from build123d import *

# Parameters (mm, degrees)
SKETCH1_W                  = 380
SKETCH1_H                  = 150
BOSS_EXTRUDE1_DEPTH        = 14
CHAMFER1_SIZE              = 1
SKETCH2_R                  = 20
CUT_EXTRUDE1_DEPTH         = 409.773776067
F_8_0_8_DIAMETER_HOLE1_D   = 8
LPATTERN1_COUNT            = 2
LPATTERN1_PITCH            = 270
F_13_0_13_DIAMETER_HOLE1_D = 13
M6_TAPPED_HOLE1_D          = 5
M6_TAPPED_HOLE1_DEPTH      = 15
M6_TAPPED_HOLE1_TIP        = 1.502151548
M6_TAPPED_HOLE2_D          = 5
M6_TAPPED_HOLE2_DEPTH      = 15
M6_TAPPED_HOLE2_TIP        = 1.502151548
M6_TAPPED_HOLE3_D          = 5
M6_TAPPED_HOLE3_DEPTH      = 15
M6_TAPPED_HOLE3_TIP        = 1.502151548
M6_TAPPED_HOLE4_D          = 5
M6_TAPPED_HOLE4_DEPTH      = 15
M6_TAPPED_HOLE4_TIP        = 1.502151548


with BuildPart() as part:
    # Sketch1 → Boss-Extrude1 (new body)
    with BuildSketch(Plane.XY):
        with Locations((190, 75)):
            Rectangle(SKETCH1_W, SKETCH1_H)
    extrude(amount=BOSS_EXTRUDE1_DEPTH)

    # Chamfer1
    chamfer1_edges = [part.edges().sort_by_distance(p)[0] for p in [
        (0, 150, 7),
        (380, 150, 7),
        (380, 0, 7),
        (0, 0, 7),
    ]]
    chamfer(chamfer1_edges, length=CHAMFER1_SIZE)

    # Sketch2 → Cut-Extrude1 (cut, through all)
    with BuildSketch(Plane.XY.offset(14)):
        with Locations((55, 75)):
            Circle(SKETCH2_R)
        with Locations((325, 75)):
            Circle(SKETCH2_R)
    extrude(amount=-CUT_EXTRUDE1_DEPTH, mode=Mode.SUBTRACT)

    # Ø8.0 (8) Diameter Hole1 (through all)
    with Locations(Plane(origin=(31.5, 98.5, 14), x_dir=(1, 0, 0), z_dir=(0, 0, 1))):
        with Locations((0, 0), (47, 0), (47, -47), (0, -47)):
            f_8_0_8_diameter_hole1 = Hole(F_8_0_8_DIAMETER_HOLE1_D / 2)

    # LPattern1: Ø8.0 (8) Diameter Hole1 ×2
    with Locations(*[(i * LPATTERN1_PITCH, 0, 0) for i in range(1, LPATTERN1_COUNT)]):
        add(f_8_0_8_diameter_hole1, mode=Mode.SUBTRACT)

    # Ø13.0 (13) Diameter Hole1 (through all)
    with Locations(Plane(origin=(355, 120, 0), x_dir=(-1, 0, 0), z_dir=(0, 0, -1))):
        with Locations((0, 0), (0, -90), (330, -90), (330, 0)):
            Hole(F_13_0_13_DIAMETER_HOLE1_D / 2)

    # M6 Tapped Hole1
    with Locations(Plane(origin=(0, 0, 0), x_dir=(-1, 0, 0), z_dir=(0, -1, 0))):
        with Locations((-370, -7), (-190, -7), (-10, -7)):
            Hole(M6_TAPPED_HOLE1_D / 2, depth=M6_TAPPED_HOLE1_DEPTH)
            with Locations((0, 0, -(M6_TAPPED_HOLE1_DEPTH + M6_TAPPED_HOLE1_TIP / 2))):  # 118° drill point
                Cone(0, M6_TAPPED_HOLE1_D / 2, M6_TAPPED_HOLE1_TIP, mode=Mode.SUBTRACT)

    # M6 Tapped Hole2
    with Locations(Plane(origin=(0, 150, 0), x_dir=(1, 0, 0), z_dir=(0, 1, 0))):
        with Locations((370, -7), (190, -7), (10, -7)):
            Hole(M6_TAPPED_HOLE2_D / 2, depth=M6_TAPPED_HOLE2_DEPTH)
            with Locations((0, 0, -(M6_TAPPED_HOLE2_DEPTH + M6_TAPPED_HOLE2_TIP / 2))):  # 118° drill point
                Cone(0, M6_TAPPED_HOLE2_D / 2, M6_TAPPED_HOLE2_TIP, mode=Mode.SUBTRACT)

    # M6 Tapped Hole3
    with Locations(Plane(origin=(380, 0, 0), x_dir=(0, 0, -1), z_dir=(1, 0, 0))):
        with Locations((-7, 125), (-7, 25)):
            Hole(M6_TAPPED_HOLE3_D / 2, depth=M6_TAPPED_HOLE3_DEPTH)
            with Locations((0, 0, -(M6_TAPPED_HOLE3_DEPTH + M6_TAPPED_HOLE3_TIP / 2))):  # 118° drill point
                Cone(0, M6_TAPPED_HOLE3_D / 2, M6_TAPPED_HOLE3_TIP, mode=Mode.SUBTRACT)

    # M6 Tapped Hole4
    with Locations(Plane.ZY):
        with Locations((7, 25), (7, 125)):
            Hole(M6_TAPPED_HOLE4_D / 2, depth=M6_TAPPED_HOLE4_DEPTH)
            with Locations((0, 0, -(M6_TAPPED_HOLE4_DEPTH + M6_TAPPED_HOLE4_TIP / 2))):  # 118° drill point
                Cone(0, M6_TAPPED_HOLE4_D / 2, M6_TAPPED_HOLE4_TIP, mode=Mode.SUBTRACT)


solid = part.part
Here's how the part is built. I have some questions about the finished solid (model axes, mm). Round coordinates to 2 decimals unless told otherwise and drop trailing zeros. Order: outer loops, then holes, each group sorted by start corner. A loop starts at its lowest first (then second) coordinate and runs counter-clockwise, first axis right, second up. Notation, with made-up numbers: M -5,-17 L 22,-17 A26 cw 22,14 Z; hole C 37,64.5 d9. An arc over 180 degrees is marked long. Return JSON: item names as keys, results as strings. Group by question number.
1. If we section it at D-D on x = 325: List the corners of the cut face in (y, z) for me.
2. If we mould it in two halves opening along Y, with no side actions, what happens to faces 1 (the face through (187, 0, 7)), 2 (the face through (305.496, 98.676, 6.902)), 3 (the face through (380, 74, 7))? For each: pulls with the +Y half, pulls with the -Y half, needs draft (parallel to the pull), parting line crosses it, or undercut.
3. I'm going to push flat-ended pins straight in: pin 1 Ø3 at (x, z) = (10, 7) entering from +Y; pin 2 Ø4.5 at (y, z) = (125, 7) entering from -X; pin 3 Ø4.5 at (x, z) = (370, 7) entering from -Y; pin 4 Ø15 at (x, y) = (25, 120) entering from +Z. Where does each tip first touch, or does it pass through?
4. If we section it at B-B on x = 55.5: List the corners of the cut face in (y, z) for me, then the cut area to 3 significant figures.
5. If we section it at A-A on y = 51.5: List the corners of the cut face in (x, z) for me, then the cut area to 3 significant figures.
6. Please list where these lines run through material, in increasing order: probe 1 along X at (y, z) = (121, 2.5); probe 2 along Y at (x, z) = (21, 10.5); probe 3 along X at (y, z) = (87, 4.25).
7. If we section it at C-C on y = 82.5: List the corners of the cut face in (x, z) for me.
Reply:
{
 "1": {"outline": "M 0,0 L 55,0 L 55,14 L 0,14 Z; M 95,0 L 150,0 L 150,14 L 95,14 Z"},
 "2": {"face 1": "pulls with the -Y half", "face 2": "undercut", "face 3": "needs draft"},
 "3": {"pin 1": "y = 134.4", "pin 2": "x = 15.15", "pin 3": "y = 15.15", "pin 4": "z = 14"},
 "4": {"outline": "M 0,0 L 55.01,0 L 55.01,14 L 0,14 Z; M 94.99,0 L 150,0 L 150,14 L 94.99,14 Z", "area": "1,540 mm^2"},
 "5": {"outline": "M 0,0 L 27.5,0 L 27.5,14 L 0,14 Z; M 35.5,0 L 74.5,0 L 74.5,14 L 35.5,14 Z; M 82.5,0 L 297.5,0 L 297.5,14 L 82.5,14 Z; M 305.5,0 L 344.5,0 L 344.5,14 L 305.5,14 Z; M 352.5,0 L 380,0 L 380,14 L 352.5,14 Z", "area": "4,870 mm^2"},
 "6": {"probe 1": "0 to 18.58, 31.42 to 348.58, 361.42 to 380", "probe 2": "0 to 24.88, 35.12 to 114.88, 125.12 to 150", "probe 3": "0 to 39, 71 to 309, 341 to 380"},
 "7": {"outline": "M 0,0 L 36.46,0 L 36.46,14 L 0,14 Z; M 73.54,0 L 306.46,0 L 306.46,14 L 73.54,14 Z; M 343.54,0 L 380,0 L 380,14 L 343.54,14 Z"}
}
